The model under review builds one solid part; all positions refer to its coordinate system, in mm. Give positions to 0.01 mm unless a question says otherwise; leave off trailing zeros. Order: outer loops, then holes, each group sorted by start corner. A loop starts at its lowest first (then second) coordinate and runs counter-clockwise, first axis right, second up. Notation, with made-up numbers: (52.5, 51) - (92.5, 51) arc R15 cw to (92.5, 70) - close; hole circle Ø9 at (81, 82). An arc over 180 degrees is marked (long way). Use CSV: the item, a comma, the result in double quotes. Start each with the question number.
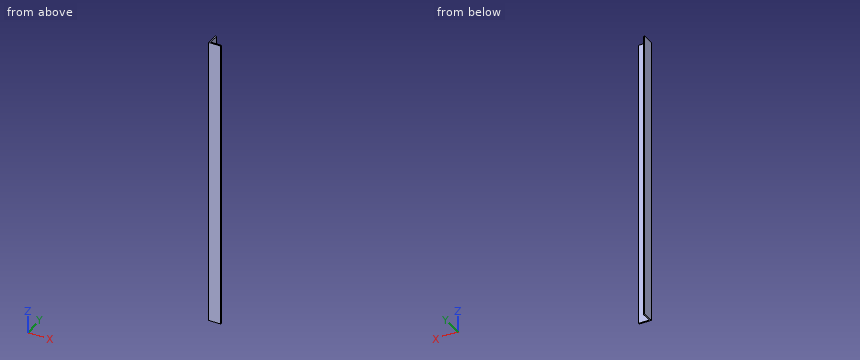
```python
from build123d import *

# Parameters (mm, degrees)
EXTRUDE1_DEPTH = 1066.8


with BuildPart() as part:
    # Sketch1 → Extrude1 (new body)
    with BuildSketch(Plane.XY):
        Polygon((-24.649517418, 21.952701214), (-24.649517418, -23.047298786), (20.350482582, -23.047298786), (20.350482582, -18.047298786), (-19.649517418, -18.047298786), (-19.649517418, 21.952701214), align=None)
    extrude(amount=EXTRUDE1_DEPTH)


solid = part.part
```
1. Consider section C-C (y = 2). Give the boundary of the cut face in (x, z).
2. Consider section B-B (z = 631.5). Give the boundary of the cut face in (x, y).
3. To check wall thickness, follow L1, parallel to X at y = -17, z = 847; L2, parallel to Y at x = 13, z = 388.5. State the ranges of each line that lie inside material, in increasing order. Write a range as [from, to].
4. Consider section A-A (x = -7). Give the boundary of the cut face in (y, z), and give its area (3 significant figures).
5. Clearance check with flat-ended pins moving along their axes: pin 1 (2 mm diameter, centred on x = -4, z = 785.5, fed in from +Y); pin 2 (8 mm diameter, centred on y = 3.5, z = 913.5, fed in from +X). State where each tip first meets the part, or that it passes through.
Answers follow:
1,outline,"(-24.65, 0) - (-19.65, 0) - (-19.65, 1066.8) - (-24.65, 1066.8) - close"
2,outline,"(-24.65, -23.05) - (20.35, -23.05) - (20.35, -18.05) - (-19.65, -18.05) - (-19.65, 21.95) - (-24.65, 21.95) - close"
3,L1,"x = [-24.65, -19.65]"
3,L2,"y = [-23.05, -18.05]"
4,outline,"(-23.05, 0) - (-18.05, 0) - (-18.05, 1066.8) - (-23.05, 1066.8) - close"
4,area,"5,330 mm^2"
5,pin 1,"stops at y = -18.05"
5,pin 2,"stops at x = -19.65"
